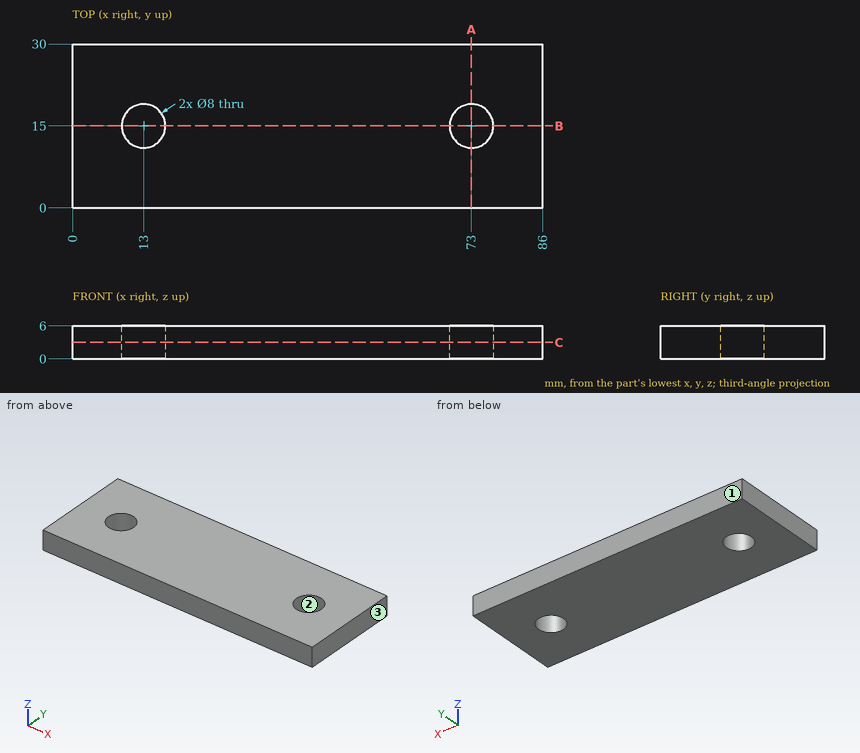
Geometry: see drawing. Coordinates: mm, zero at the bounding-box minimum. Coordinates: 2 decimals unless noted, no trailing zeros. Order: outer loops, then holes, each group sorted by start corner. A loop starts at its lowest first (then second) coordinate and runs counter-clockwise, first axis right, second up. Notation, with made-up numbers: (22.5, -31) - (73.5, -31) arc R29 cw to (73.5, 1) - close; hole circle Ø9 at (-11, 61). An arc over 180 degrees is marked (long way). Use one line per item in the form item = value.
1) Ray query, L1, parallel to Y at x = 13, z = 4.2; L2, parallel to X at y = 16.25, z = 3.55; L3, parallel to X at y = 14.5, z = 4.85. Return the intervals inside material, ascending.
Solutions:
L1 = 0 to 11, 19 to 30
L2 = 0 to 9.2, 16.8 to 69.2, 76.8 to 86
L3 = 0 to 9.03, 16.97 to 69.03, 76.97 to 86
2) Section A-A (x = 73). Return loops of the section in (y, z), then the cut area to 3 significant figures.
Solutions:
outline = (0, 0) - (11, 0) - (11, 6) - (0, 6) - close; (19, 0) - (30, 0) - (30, 6) - (19, 6) - close
area = 132 mm^2
3) Section B-B (y = 15). Return loops of the section in (x, z).
Solutions:
outline = (0, 0) - (9, 0) - (9, 6) - (0, 6) - close; (17, 0) - (69, 0) - (69, 6) - (17, 6) - close; (77, 0) - (86, 0) - (86, 6) - (77, 6) - close
4) Section C-C (z = 3). Return loops of the section in (x, y).
Solutions:
outline = (0, 0) - (86, 0) - (86, 30) - (0, 30) - close; hole circle Ø8 at (13, 15); hole circle Ø8 at (73, 15)
5) Mould query, pull axis X, two halves, no side actions, for the marked faces 1, 2 and 3. Classes: +X half, -X half, draft (parallel to the pull), parting line (faces both ways), or undercut.
Solutions:
face_1 = draft
face_2 = undercut
face_3 = +X half
